Could you check a few things on this model? Use its own coordinates, in mm. Round coordinates to 2 decimals unless told otherwise and drop trailing zeros. Order: outer loops, then holes, each group sorted by start corner. A loop starts at its lowest first (then second) coordinate and runs counter-clockwise, first axis right, second up. Notation, with made-up numbers: (49, -3.5) - (76, -3.5) arc R20 ccw to (76, 9.5) - close; hole circle Ø5 at (-31, 29). An arc over 180 degrees is marked (long way). Return JSON: item names as keys, results as strings. Group by question number.
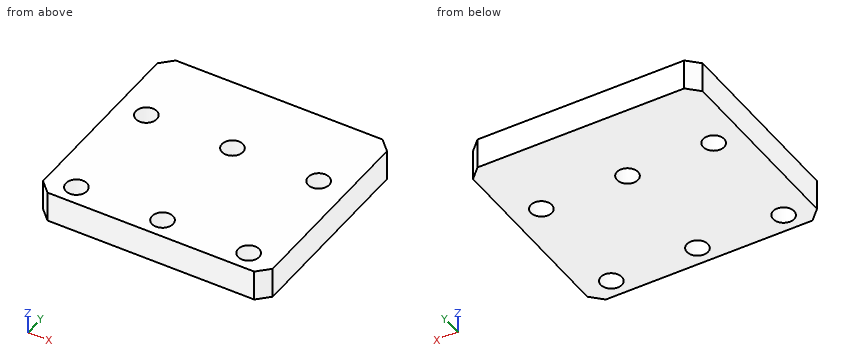
from build123d import *

# Parameters (mm, degrees)
SKETCH1_W                  = 60
SKETCH1_H                  = 55
BOSS_EXTRUDE1_DEPTH        = 8
F_5_5_5_5_DIAMETER_HOLE1_D = 5.5
CHAMFER1_SIZE              = 3


with BuildPart() as part:
    # Sketch1 → Boss-Extrude1 (new body)
    with BuildSketch(Plane.XY):
        Rectangle(SKETCH1_W, SKETCH1_H)
    extrude(amount=BOSS_EXTRUDE1_DEPTH)

    # Ø5.5 (5.5) Diameter Hole1 (through all)
    with Locations(Plane.XY.offset(8)):
        with Locations((-22.5, -22.5), (-22.5, 7.5), (0, 7.5), (0, -22.5), (22.5, -22.5), (22.5, 7.5)):
            Hole(F_5_5_5_5_DIAMETER_HOLE1_D / 2)

    # Chamfer1
    chamfer1_edges = [part.edges().sort_by_distance(p)[0] for p in [
        (30, -27.5, 4),
        (-30, -27.5, 4),
        (-30, 27.5, 4),
        (30, 27.5, 4),
    ]]
    chamfer(chamfer1_edges, length=CHAMFER1_SIZE)


solid = part.part
1) If I drill on line 1 along Y through (x, z) = (22.5, 4.5); line 2 along X through (y, z) = (-20, 2.5); line 3 along X through (y, z) = (-24, 6.5), over which ranges is the centre line in solid material (lowest first)? Write a range as from..to.
2) I want a section at C-C, the plane z = 2. List the corners of the cut face in (x, y) for me, plus the area to 3 significant figures.
3) I want a section at B-B, the plane x = 0. List the corners of the cut face in (y, z) for me, plus the area to 3 significant figures.
4) I want a section at D-D, the plane x = 22. List the corners of the cut face in (y, z) for me.
5) Will this pin go through, and if not, where does the flat tip stop? pin 1 (5 mm diameter, centred on x = -22.5, y = -22.5, fed in from -Z).
6) I want a section at A-A, the plane y = -22.5. List the corners of the cut face in (x, z) for me, plus the area to 3 significant figures.
Outcome:
{
 "1": {"line 1": "-27.5..-25.25, -19.75..4.75, 10.25..27.5", "line 2": "-30..-23.65, -21.35..-1.15, 1.15..21.35, 23.65..30", "line 3": "-30..-24.8, -20.2..-2.3, 2.3..20.2, 24.8..30"},
 "2": {"outline": "(-30, -24.5) - (-27, -27.5) - (27, -27.5) - (30, -24.5) - (30, 24.5) - (27, 27.5) - (-27, 27.5) - (-30, 24.5) - close; hole circle Ø5.5 at (-22.5, -22.5); hole circle Ø5.5 at (-22.5, 7.5); hole circle Ø5.5 at (0, -22.5); hole circle Ø5.5 at (0, 7.5); hole circle Ø5.5 at (22.5, -22.5); hole circle Ø5.5 at (22.5, 7.5)", "area": "3,140 mm^2"},
 "3": {"outline": "(-27.5, 0) - (-25.25, 0) - (-25.25, 8) - (-27.5, 8) - close; (-19.75, 0) - (4.75, 0) - (4.75, 8) - (-19.75, 8) - close; (10.25, 0) - (27.5, 0) - (27.5, 8) - (10.25, 8) - close", "area": "352 mm^2"},
 "4": {"outline": "(-27.5, 0) - (-25.2, 0) - (-25.2, 8) - (-27.5, 8) - close; (-19.8, 0) - (4.8, 0) - (4.8, 8) - (-19.8, 8) - close; (10.2, 0) - (27.5, 0) - (27.5, 8) - (10.2, 8) - close"},
 "5": {"pin 1": "through"},
 "6": {"outline": "(-30, 0) - (-25.25, 0) - (-25.25, 8) - (-30, 8) - close; (-19.75, 0) - (-2.75, 0) - (-2.75, 8) - (-19.75, 8) - close; (2.75, 0) - (19.75, 0) - (19.75, 8) - (2.75, 8) - close; (25.25, 0) - (30, 0) - (30, 8) - (25.25, 8) - close", "area": "348 mm^2"}
}
